Geometry: final body of the model. Coordinates: model frame, mm. A direction names the side the tool comes from. Coordinates: 2 decimals unless noted, no trailing zeros. Order: outer loops, then holes, each group sorted by start corner. A loop starts at its lowest first (then second) coordinate and runs counter-clockwise, first axis right, second up. Notation, with made-up numbers: (43.5, 18.25) -> (67.5, 18.25) arc R26 ccw to (67.5, 43.25) -> close; hole circle Ø1 at (22, -18). An arc over 180 degrees is marked (long way). Answer in a Markdown table with one row per item. Add a question column.
1) Section query A-A on y = 11. Return the cut outline in (x, z).
2) Ray query, line 1 (Y direction, x = 5.5, z = 22); line 2 (Z direction, x = -25, y = 20.5); line 3 (Z direction, x = 38.5, y = 19.5). Return the intervals inside material, ascending. Write a range as from..to.
3) Pull-direction query (Y, two-part tool) for faces 1 (the face through (-31, 16, 30)), 2 (the face through (-27, 28, 20)), 3 (the face through (-20, 0, 27)); classes: +Y half, -Y half, draft (parallel to the pull), parting line (faces both ways), or undercut.
4) Contact query for flat-ended pins moving along their axis: P1, Ø8, axis at x = 24.5, z = -27.5, coming from the -Y side; P2, Ø11.5, axis at x = 2, z = 14.5, coming from the -Y side; P3, Ø1, axis at y = -21.5, z = -0.5, coming from the +X side; P4, Ø2.5, axis at x = 20, y = 27, coming from the +Z side. Output: stop coordinate, or through.
5) Section query D-D on y = 2.5. Return the cut outline in (x, z), then the cut area to 3 significant figures.
6) Section query B-B on z = 28.5. Return the cut outline in (x, y), then the cut area to 3 significant figures.
7) Section query C-C on x = 47. Return the cut outline in (y, z).
8) Set-up query: faces 4 (the face through (-9, 28, -20)), 5 (the face through (-20.31, -10.831, 12.253)), 6 (the face through (-75, 5, 1)), 7 (the face through (33.55, -7.4, -1.27)), 8 (the face through (-5, 16, -30)). Return all of +Z, -Z, +X, -X, +Y, -Y with unobstructed straight access to the full face (end or side cutting, diameter ignored); none if empty.
```python
from build123d import *

# Parameters (mm, degrees)
BASE_BLOCK_150X85X32_DEPTH = 32
T_SLOT_CUT_DEPTH           = 160.154798859
T_SLOT_CUT_DEPTH_BACK      = 160.154798859
TAPERED_FOOT_BOSS_DEPTH    = 40
FOOT_RELIEF_CUT_DEPTH      = 101.347613869
FOOT_RELIEF_CUT_DEPTH_BACK = 101.347613869
FOOT_RELIEF_SKETCH_R       = 10


with BuildPart() as part:
    # Base Block Sketch → Base Block 150x85x32 (new body)
    with BuildSketch(Plane(origin=(0, 0, 0), x_dir=(1, 0, 0), z_dir=(0, 1, 0))):
        Polygon((-75, 42.5), (75, 42.5), (0, -42.5), (-75, -42.5), align=None)
    extrude(amount=BASE_BLOCK_150X85X32_DEPTH)

    # T-Slot Sketch → T-Slot Cut (cut, two sides: drawn at the far end of the back side and taken through both)
    with BuildSketch(Plane.ZY.offset(75).offset(-T_SLOT_CUT_DEPTH_BACK)):
        Polygon((-20, 32), (-20, 24), (-30, 24), (-30, 8), (30, 8), (30, 24), (20, 24), (20, 32), align=None)
    extrude(amount=T_SLOT_CUT_DEPTH + T_SLOT_CUT_DEPTH_BACK, mode=Mode.SUBTRACT)

    # Tapered Foot Sketch → Tapered Foot Boss (add)
    with BuildSketch(Plane.XZ):
        Polygon((-75, 10.790645392), (-73.43565535, 20.667528798), (34.323374911, 3.6001751), (32.759030261, -6.276708306), align=None)
    extrude(amount=TAPERED_FOOT_BOSS_DEPTH)

    # Foot Relief Sketch → Foot Relief Cut (cut, two sides: drawn at the far end of the back side and taken through both)
    with BuildSketch(Plane(origin=(1.396210415, 0, 8.815325621), x_dir=(0.9876883405951378, 0, -0.15643446504023126), z_dir=(0.15643446504023126, 0, 0.9876883405951378)).offset(-FOOT_RELIEF_CUT_DEPTH_BACK)):
        Polygon((33.337605744, -15), (8.337605744, -40), (33.337605744, -40), align=None)
        with Locations((-25.764654384, -22)):
            Circle(FOOT_RELIEF_SKETCH_R)
        Polygon((-52.670643616, -40), (-75.764654384, 0), (-75.764654384, -40), align=None)
    extrude(amount=FOOT_RELIEF_CUT_DEPTH + FOOT_RELIEF_CUT_DEPTH_BACK, mode=Mode.SUBTRACT)


solid = part.part
```
Result:
| question | item | result |
|---|---|---|
| 1 | outline | (-75, -42.5) -> (75, -42.5) -> (63.97, -30) -> (-75, -30) -> close; (-75, 30) -> (11.03, 30) -> (0, 42.5) -> (-75, 42.5) -> close |
| 2 | line 1 | 0..8, 24..32 |
| 2 | line 2 | -42.5..-30, 30..42.5 |
| 2 | line 3 | -42.5..-30 |
| 3 | face 1 | undercut |
| 3 | face 2 | draft |
| 3 | face 3 | -Y half |
| 4 | P1 | y = 0 |
| 4 | P2 | y = -40 |
| 4 | P3 | x = 27.61 |
| 4 | P4 | z = 21.25 |
| 5 | outline | (-75, -42.5) -> (75, -42.5) -> (0, 42.5) -> (-75, 42.5) -> close |
| 5 | area | 9,560 mm2 |
| 6 | outline | (-75, 0) -> (12.35, 0) -> (12.35, 8) -> (-75, 8) -> close; (-75, 24) -> (12.35, 24) -> (12.35, 32) -> (-75, 32) -> close |
| 6 | area | 1,400 mm2 |
| 7 | outline | (0, -42.5) -> (32, -42.5) -> (32, -20) -> (24, -20) -> (24, -30) -> (8, -30) -> (8, -10.77) -> (0, -10.77) -> close |
| 8 | face 4 | +X, -X, +Y |
| 8 | face 5 | +Z, +X, -Y |
| 8 | face 6 | +Z, -Z, -X, +Y, -Y |
| 8 | face 7 | -Z, +X, -Y |
| 8 | face 8 | +X, -X |
